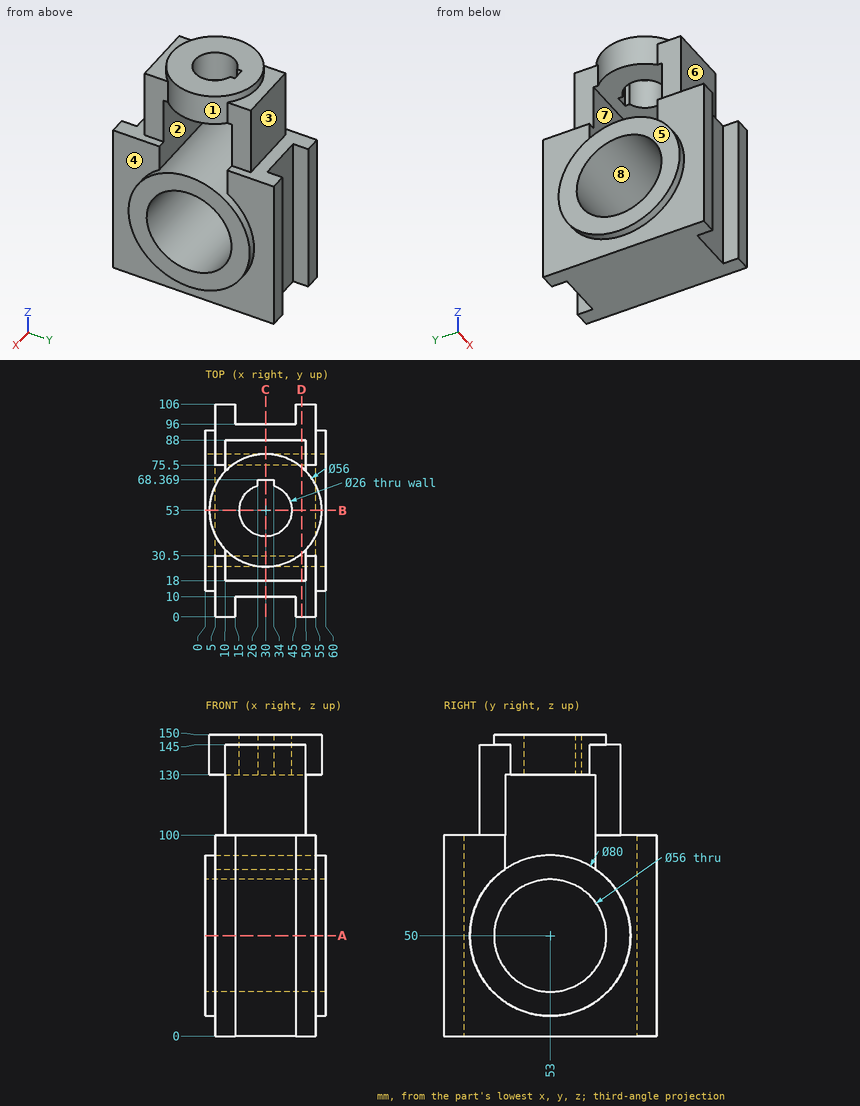
Print and shaded views of the part. All mm, measured from the part's lowest x, y and z. A direction names the side the tool comes from. Coordinates: 2 decimals unless noted, no trailing zeros. Write each loop counter-clockwise with the first axis right and the second up, starting at its lowest first coordinate (ties: lowest second). Pieces come first, ordered by that corner, then holes. Notation, with made-up numbers: M 48.5,-7 L 60.5,-7 A29 cw 60.5,17 Z; hole C 32,45.5 d2. An arc over 180 degrees is marked long. Return JSON: item names as keys, results as strings.
1. Saw through at C-C, the plane x = 30. Write the cut outline in (y, z), then the cut area to 3 significant figures.
Determined:
{"outline": "M 10,0 L 96,0 L 96,100 L 88,100 L 88,145 L 81,145 L 81,150 L 68.37,150 L 68.37,130 L 75.5,130 L 75.5,83.07 A40 ccw 30.5,83.07 L 30.5,130 L 40,130 L 40,150 L 25,150 L 25,145 L 18,145 L 18,100 L 10,100 Z; hole C 53,50 d56", "area": "7,100 mm²"}
2. Probe L1, parallel to Y at x = 30, z = 146.25; L2, parallel to X at y = 53, z = 142; L3, parallel to Y at x = 16, z = 50. List the from-to ranges inside material, lowest first.
Determined:
{"L1": "25 to 40, 68.37 to 81", "L2": "2 to 17, 43 to 58", "L3": "10 to 25, 81 to 96"}
3. Pull direction Y, two halves, no side cores. Call the marked faces 5, 6, 7 and 8: pulls with the +Y half, pulls with the -Y half, needs draft (parallel to the pull), parting line crosses it, or undercut.
Determined:
{"face 5": "needs draft", "face 6": "pulls with the -Y half", "face 7": "undercut", "face 8": "undercut"}
4. Saw through at D-D, the plane x = 48. Write the cut outline in (y, z), then the cut area to 3 significant figures.
Determined:
{"outline": "M 0,0 L 106,0 L 106,100 L 88,100 L 88,145 L 74.45,145 L 74.45,150 L 31.55,150 L 31.55,145 L 18,145 L 18,100 L 0,100 Z; hole C 53,50 d56; hole M 30.5,83.07 A40 cw 75.5,83.07 L 75.5,130 L 30.5,130 Z", "area": "9,600 mm²"}
5. Saw through at A-A, the plane z = 50. Write the cut outline in (x, y).
Determined:
{"outline": "M 0,13 L 5,13 L 5,0 L 15,0 L 15,10 L 45,10 L 45,0 L 55,0 L 55,13 L 60,13 L 60,25 L 0,25 Z; M 0,81 L 60,81 L 60,93 L 55,93 L 55,106 L 45,106 L 45,96 L 15,96 L 15,106 L 5,106 L 5,93 L 0,93 Z"}
6. 3-axis set-ups, long thin cutter, end or side, ignore diameter. For the marked faces 1, 2, 3 and 4: which of +Z, -Z, +X, -X, +Y, -Y reach the whole face in a straight line?
Determined:
{"face 1": "+Z", "face 2": "+X, -X", "face 3": "+Z, +X, -X, +Y", "face 4": "+X"}
7. Flat gauge pins, fed straight in: pin 1 Ø8 at (y, z) = (5, 26.5) entering from +X; pin 2 Ø1 at (x, z) = (47, 131) entering from +Y; pin 3 Ø6.5 at (x, z) = (28, 143.5) entering from -Y; pin 4 Ø6 at (y, z) = (60.5, 125) entering from +X. Where does each tip first touch, or does it go through?
Determined:
{"pin 1": "x = 55", "pin 2": "y = 88", "pin 3": "y = 18", "pin 4": "through"}
8. Saw through at B-B, the plane y = 53. Write the cut outline in (x, z).
Determined:
{"outline": "M 0,10 L 5,10 L 5,0 L 55,0 L 55,10 L 60,10 L 60,22 L 0,22 Z; M 0,78 L 60,78 L 60,90 L 0,90 Z; M 2,130 L 17,130 L 17,150 L 2,150 Z; M 43,130 L 58,130 L 58,150 L 43,150 Z"}
